Can you work these out from the model? Positions are in its coordinate system, mm. Give positions to 0.01 mm unless a question says otherwise; leave off trailing zeros. Write each loop counter-clockwise with the first axis right and the second up, starting at its lowest first coordinate (ties: lowest second). Pieces come first, ordered by that corner, then holes.
1. If I drill on probe 1 along Y at (x, z) = (-80, 3); probe 2 along Y at (x, z) = (16.5, 2.7), over which ranges is the centre line in solid material (lowest first)?
2. I'm going to push flat-ended pins straight in: pin 1 (6.5 mm diameter, centred on x = 20, y = -70, fed in from -Z); pin 2 (5 mm diameter, centred on x = -73.5, y = 23, fed in from -Z). Where does each tip first touch, or does it pass through?
3. Suppose I cut it at B-B (y = 70). Please give me the cut outline in (x, z), and give its area (3 significant figures).
4. Suppose I cut it at A-A (x = 20). Please give me the cut outline in (y, z), and give its area (3 significant figures).
```python
from build123d import *

# Parameters (mm, degrees)
SKETCH_1_W          = 240
SKETCH_1_H          = 208
EXTRUDE_1_DEPTH     = 4
SKETCH_2_R          = 5.5
CUT_EXTRUDE_1_DEPTH = 10


with BuildPart() as part:
    # 草图1 → 凸台-拉伸1 (new body)
    with BuildSketch(Plane.XY):
        Rectangle(SKETCH_1_W, SKETCH_1_H)
    extrude(amount=EXTRUDE_1_DEPTH)

    # 草图2 → 切除-拉伸1 (cut)
    with BuildSketch(Plane(origin=(0, 0, 0), x_dir=(-1, 0, 0), z_dir=(0, 0, -1))):
        with Locations((-20, -70)):
            Circle(SKETCH_2_R)
        with Locations((80, -70)):
            Circle(SKETCH_2_R)
        with Locations((80, 70)):
            Circle(SKETCH_2_R)
        with Locations((-20, 70)):
            Circle(SKETCH_2_R)
    extrude(amount=-CUT_EXTRUDE_1_DEPTH, mode=Mode.SUBTRACT)


solid = part.part
```
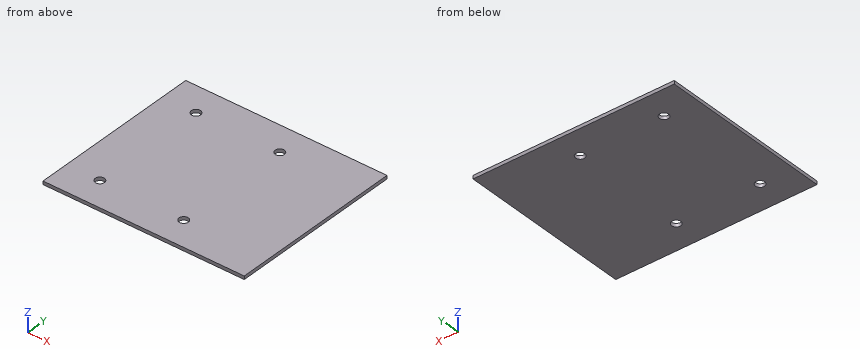
Checks:
1. probe 1: y = -104 to -75.5, -64.5 to 64.5, 75.5 to 104
1. probe 2: y = -104 to -74.24, -65.76 to 65.76, 74.24 to 104
2. pin 1: passes through
2. pin 2: stops at z = 0
3. outline: (-120, 0) - (-85.5, 0) - (-85.5, 4) - (-120, 4) - close; (-74.5, 0) - (14.5, 0) - (14.5, 4) - (-74.5, 4) - close; (25.5, 0) - (120, 0) - (120, 4) - (25.5, 4) - close
3. area: 872 mm2
4. outline: (-104, 0) - (-75.5, 0) - (-75.5, 4) - (-104, 4) - close; (-64.5, 0) - (64.5, 0) - (64.5, 4) - (-64.5, 4) - close; (75.5, 0) - (104, 0) - (104, 4) - (75.5, 4) - close
4. area: 744 mm2
